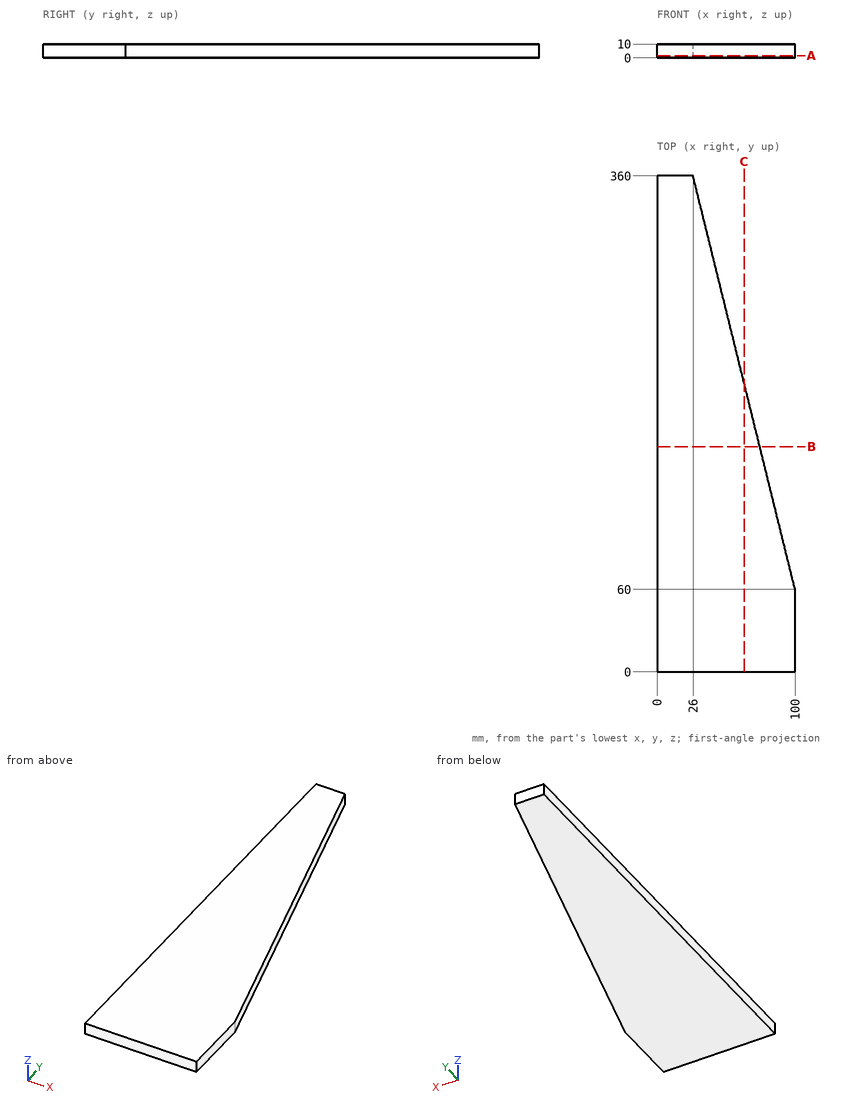
Design review of the part shown in the three views and the two pictorial views. Dimensions are in mm from the part's minimum x, y and z. Coordinates: 2 decimals unless noted, no trailing zeros. Order: outer loops, then holes, each group sorted by start corner. A loop starts at its lowest first (then second) coordinate and runs counter-clockwise, first axis right, second up.
Item 1: For pin 1 Ø3 at (y, z) = (90, 6.5) entering from +X, flat-tipped, find the tip position at first contact; note if it passes through.
Item 2: Take a section at C-C, the plane x = 63. Write out the cut boundary in (y, z).
Item 3: For line 1 (X direction, y = 107, z = 5.5); line 2 (X direction, y = 253.5, z = 3.5), list the stretches that pass through material, from the lowest coordinate up.
Item 4: Take a section at B-B, the plane y = 163.5. Write out the cut boundary in (x, z), then the cut area to 3 significant figures.
Item 5: Take a section at A-A, the plane z = 1.5. Write out the cut boundary in (x, y).
The answers:
1. pin 1: stops at x = 92.97
2. outline: (0, 0) - (210, 0) - (210, 10) - (0, 10) - close
3. line 1: x = 0 to 88.41
3. line 2: x = 0 to 52.27
4. outline: (0, 0) - (74.47, 0) - (74.47, 10) - (0, 10) - close
4. area: 745 mm2
5. outline: (0, 0) - (100, 0) - (100, 60) - (26, 360) - (0, 360) - close
